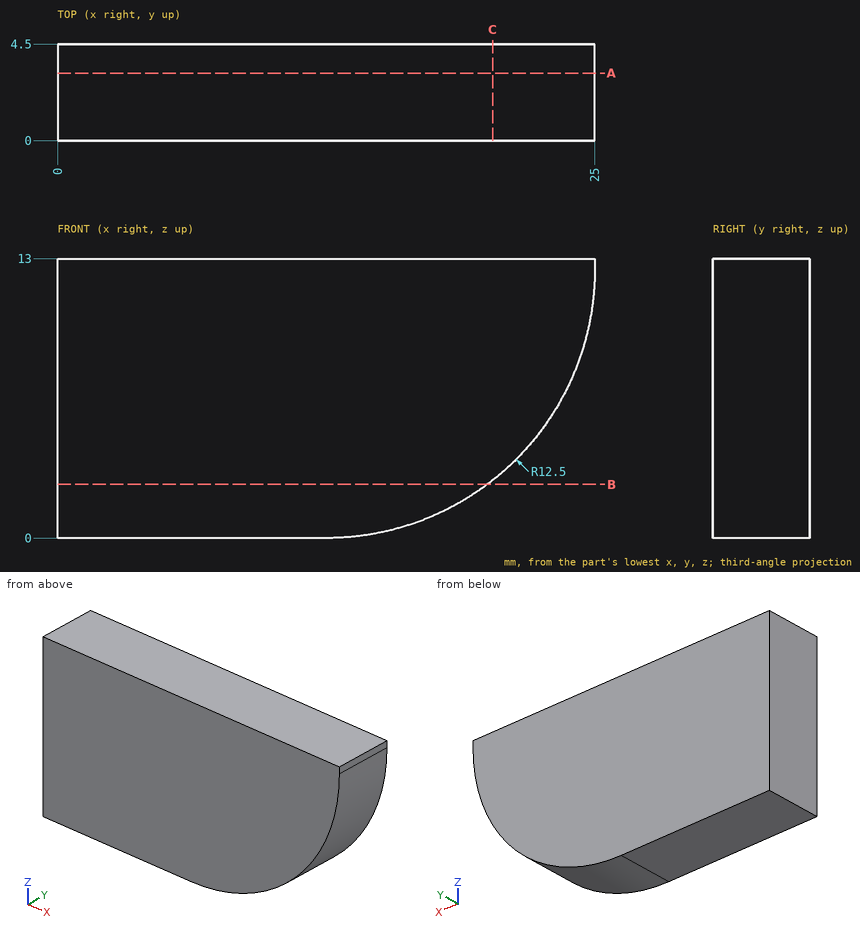
Drawing for the job (mm, zero at the part's lowest x, y, z). Give positions to 0.01 mm unless a question says otherwise; leave off trailing zeros. Order: outer loops, then holes, each group sorted by start corner. A loop starts at its lowest first (then second) coordinate and runs counter-clockwise, first axis right, second up. Notation, with made-up numbers: (-23.75, -33.75) -> (-0.75, -33.75) arc R25 ccw to (-0.75, -10.75) -> close; hole circle Ø10 at (-24, -24.5). An arc over 180 degrees is marked (long way). Use one line per item in the form item = value.
(1) Saw through at B-B (z = 2.5). Write the cut outline in (x, y).
Solution:
outline = (0, 0) -> (20, 0) -> (20, 4.5) -> (0, 4.5) -> close
(2) Drill centre lines: line 1 (X direction, y = 0.65, z = 9); line 2 (X direction, y = 0.35, z = 10.25); line 3 (Z direction, x = 14.25, y = 0.6). Where is each one in solid material? Low to high. Write a range as from..to.
Solution:
line_1 = 0..24.5
line_2 = 0..24.8
line_3 = 0.12..13
(3) Saw through at A-A (y = 3.15). Write the cut outline in (x, z), then the cut area to 3 significant figures.
Solution:
outline = (0, 0) -> (12.5, 0) arc R12.5 ccw to (25, 12.5) -> (25, 13) -> (0, 13) -> close
area = 291 mm²
(4) Saw through at C-C (x = 20.25). Write the cut outline in (y, z).
Solution:
outline = (0, 2.69) -> (4.5, 2.69) -> (4.5, 13) -> (0, 13) -> close
